```python
from build123d import *

# Parameters (mm, degrees)
SKETCH1_W                                        = 45
SKETCH1_H                                        = 20
BOSS_EXTRUDE1_DEPTH                              = 30
CUT_EXTRUDE1_DEPTH                               = 56
CUT_EXTRUDE1_DEPTH_BACK                          = 56
SKETCH2_W                                        = 5
SKETCH2_H                                        = 4
CHAMFER1_SIZE                                    = 8
HOLE_FOR_SOCKET_HEAD_CAP_SCREW_TYPE1_D           = 4.5
HOLE_FOR_SOCKET_HEAD_CAP_SCREW_TYPE1_CBORE_D     = 8
HOLE_FOR_SOCKET_HEAD_CAP_SCREW_TYPE1_CBORE_DEPTH = 4.6
CUT_EXTRUDE2_DEPTH                               = 56
CUT_EXTRUDE2_DEPTH_BACK                          = 56
SKETCH7_W                                        = 10
SKETCH7_H                                        = 2


with BuildPart() as part:
    # Sketch1 → Boss-Extrude1 (new body)
    with BuildSketch(Plane.XY):
        Rectangle(SKETCH1_W, SKETCH1_H)
    extrude(amount=BOSS_EXTRUDE1_DEPTH)

    # Sketch2 → Cut-Extrude1 (cut, two sides: drawn at the far end of the back side and taken through both)
    with BuildSketch(Plane.ZY.offset(22.5).offset(-CUT_EXTRUDE1_DEPTH_BACK)):
        Polygon((0, -2), (15, -2), (20, 10), (0, 10), align=None)
        with Locations((27.5, 4)):
            Rectangle(SKETCH2_W, SKETCH2_H)
    extrude(amount=CUT_EXTRUDE1_DEPTH + CUT_EXTRUDE1_DEPTH_BACK, mode=Mode.SUBTRACT)

    # Chamfer1
    chamfer1_edges = [part.edges().sort_by_distance(p)[0] for p in [
        (0, -10, 30),
    ]]
    chamfer(chamfer1_edges, length=CHAMFER1_SIZE)

    # Hole for socket head cap screw, type1 (through all)
    with Locations(Plane(origin=(0, -2, 0), x_dir=(1, 0, 0), z_dir=(0, 1, 0))):
        with Locations((-12.5, -5), (12.5, -5)):
            CounterBoreHole(HOLE_FOR_SOCKET_HEAD_CAP_SCREW_TYPE1_D / 2, HOLE_FOR_SOCKET_HEAD_CAP_SCREW_TYPE1_CBORE_D / 2, HOLE_FOR_SOCKET_HEAD_CAP_SCREW_TYPE1_CBORE_DEPTH)

    # Sketch7 → Cut-Extrude2 (cut, two sides: drawn at the far end of the back side and taken through both)
    with BuildSketch(Plane.ZY.offset(22.5).offset(-CUT_EXTRUDE2_DEPTH_BACK)):
        with Locations((5, -9)):
            Rectangle(SKETCH7_W, SKETCH7_H)
    extrude(amount=CUT_EXTRUDE2_DEPTH + CUT_EXTRUDE2_DEPTH_BACK, mode=Mode.SUBTRACT)


solid = part.part
```
Model file for the job. Use its own axes, mm. A direction names the side the tool comes from. Coordinates: 2 decimals unless noted, no trailing zeros. Write each loop counter-clockwise with the first axis right and the second up, starting at its lowest first coordinate (ties: lowest second). Pieces come first, ordered by that corner, then holes. Notation, with made-up numbers: (1, 53.25) - (57, 53.25) arc R16 cw to (57, 63.25) - close; hole circle Ø11 at (33.25, 64.5). An arc over 180 degrees is marked (long way). Use a Markdown table: item, result. Add a question column.
Item 1: Drop flat-ended pins along their axis: pin 1 (9 mm diameter, centred on x = 11.5, z = 7, fed in from +Y); pin 2 (8 mm diameter, centred on x = -6, z = 3.5, fed in from -Y); pin 3 (4.5 mm diameter, centred on x = -1.5, y = 3.5, fed in from +Z); pin 4 (5 mm diameter, centred on x = 12.5, z = 5, fed in from +Y). Give the stop position or say it passes through.
Item 2: Drill centre lines: line 1 along X through (y, z) = (-4.25, 7); line 2 along Y through (x, z) = (-5.5, 8.25); line 3 along Z through (x, y) = (-12.5, -7.55). Where is each one in solid material? Low to high.
Item 3: Band-saw the part on A-A, the plane z = 5. Write the cut outline in (x, y).
Item 4: Band-saw the part on D-D, the plane y = -4.75. Write the cut outline in (x, z), and give its area (3 significant figures).
Item 5: Band-saw the part on C-C, the plane x = -12.5. Write the cut outline in (y, z).
Item 6: 3-axis set-ups, long thin cutter, end or side, ignore diameter. For faces 4 (the face through (-11, -6.6, 7)), 5 (the face through (0, -8, 5)), 6 (the face through (0, -2, 7)): which of +Z, -Z, +X, -X, +Y, -Y reach the whole face in a straight line?
Item 7: Band-saw the part on B-B, the plane z = 27.5. Write the cut outline in (x, y), and give its area (4 significant figures).
Item 8: Two-plate mould, pull along Z, no slides. Class faces 1 (the face through (-10.252, -7.31, 4.901)), 2 (the face through (0, 4, 25)), 3 (the face through (0, 10, 25)): pulls with the +Z half, pulls with the -Z half, needs draft (parallel to the pull), parting line crosses it, or undercut.
A:
| question | item | result |
|---|---|---|
| 1 | pin 1 | stops at y = -2 |
| 1 | pin 2 | stops at y = -8 |
| 1 | pin 3 | stops at z = 30 |
| 1 | pin 4 | stops at y = -6.6 |
| 2 | line 1 | x = -22.5 to -15.96, -9.04 to 9.04, 15.96 to 22.5 |
| 2 | line 2 | y = -8 to -2 |
| 2 | line 3 | z = 0 to 2.75, 7.25 to 24.45 |
| 3 | outline | (-22.5, -8) - (-14.75, -8) - (-14.75, -6.6) - (-16.5, -6.6) - (-16.5, -2) - (-22.5, -2) - close; (-10.25, -8) - (10.25, -8) - (10.25, -6.6) - (8.5, -6.6) - (8.5, -2) - (-8.5, -2) - (-8.5, -6.6) - (-10.25, -6.6) - close; (14.75, -8) - (22.5, -8) - (22.5, -2) - (16.5, -2) - (16.5, -6.6) - (14.75, -6.6) - close |
| 4 | outline | (-22.5, 0) - (22.5, 0) - (22.5, 27.25) - (-22.5, 27.25) - close; hole circle Ø8 at (-12.5, 5); hole circle Ø8 at (12.5, 5) |
| 4 | area | 1,130 mm² |
| 5 | outline | (-10, 10) - (-8, 10) - (-8, 7.25) - (-6.6, 7.25) - (-6.6, 9) - (-2, 9) - (-2, 15) - (10, 20) - (10, 30) - (6, 30) - (6, 25) - (2, 25) - (2, 30) - (-2, 30) - (-10, 22) - close; (-8, 0) - (-2, 0) - (-2, 1) - (-6.6, 1) - (-6.6, 2.75) - (-8, 2.75) - close |
| 6 | face 4 | +Y |
| 6 | face 5 | -Z, +X, -X, -Y |
| 6 | face 6 | -Z, +X, -X, +Y |
| 7 | outline | (-22.5, -4.5) - (22.5, -4.5) - (22.5, 2) - (-22.5, 2) - close; (-22.5, 6) - (22.5, 6) - (22.5, 10) - (-22.5, 10) - close |
| 7 | area | 472.5 mm² |
| 8 | face 1 | undercut |
| 8 | face 2 | pulls with the +Z half |
| 8 | face 3 | needs draft |
